from build123d import *

# Parameters (mm, degrees)
SKETCH2_R           = 35
SKETCH2_R_2         = 25.5
BOSS_EXTRUDE1_DEPTH = 3
SKETCH3_R           = 4
CUT_EXTRUDE1_DEPTH  = 5
SKETCH8_W           = 8
SKETCH8_H           = 8.160533217
CUT_EXTRUDE3_DEPTH  = 50.588305073
SKETCH9_R           = 1.65
CUT_EXTRUDE4_DEPTH  = 50.588305073


with BuildPart() as part:
    # Sketch2 → Boss-Extrude1 (new body)
    with BuildSketch(Plane.XY):
        Circle(SKETCH2_R)
        Circle(SKETCH2_R_2, mode=Mode.SUBTRACT)
    extrude(amount=BOSS_EXTRUDE1_DEPTH)

    # Sketch3 → Cut-Extrude1 (cut)
    with BuildSketch(Plane(origin=(0, 0, 0), x_dir=(-1, 0, 0), z_dir=(0, 0, -1))):
        with Locations((0, -33)):
            Circle(SKETCH3_R)
    extrude(amount=-CUT_EXTRUDE1_DEPTH, mode=Mode.SUBTRACT)

    # Sketch8 → Cut-Extrude3 (cut, through all)
    with BuildSketch(Plane.XY.offset(3)):
        with Locations((0, -37.080266608)):
            Rectangle(SKETCH8_W, SKETCH8_H)
    extrude(amount=-CUT_EXTRUDE3_DEPTH, mode=Mode.SUBTRACT)

    # Sketch9 → Cut-Extrude4 (cut, through all)
    with BuildSketch(Plane.XY.offset(3)):
        with Locations((30, 0)):
            Circle(SKETCH9_R)
        with Locations(Location((-30, 0, 0), (0, 0, 180))):
            Circle(SKETCH9_R)
    extrude(amount=-CUT_EXTRUDE4_DEPTH, mode=Mode.SUBTRACT)


solid = part.part
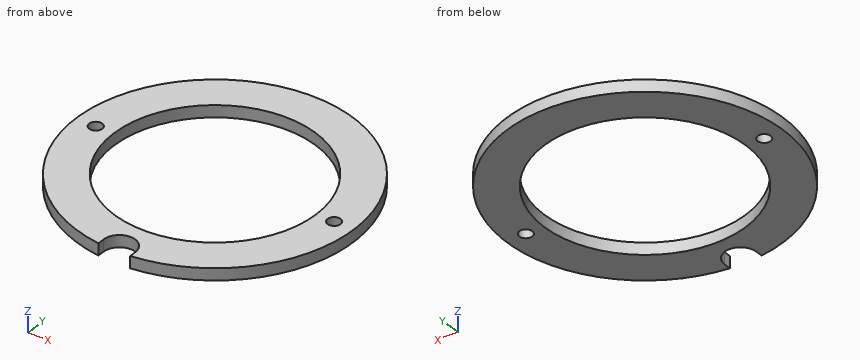
Design review of the part built by this model. Coordinates are the model's own, in mm. Round coordinates to 2 decimals unless told otherwise and drop trailing zeros. Write each loop counter-clockwise with the first axis right and the second up, starting at its lowest first coordinate (ties: lowest second). Pieces come first, ordered by that corner, then holes. Notation, with made-up numbers: (44.5, 84.25) - (94.5, 84.25) arc R23 cw to (94.5, 97.25) - close; hole circle Ø10 at (58, 86.5). An arc over 180 degrees is marked (long way). Use a Markdown table: item, result. Add a question column.
1. We need section B-B (x = 30). State the section outline as (y, z) points.
2. We need section A-A (z = 2.15). State the section outline as (x, y) points.
3. Clearance check with flat-ended pins moving along their axes: pin 1 (1 mm diameter, centred on y = -1, z = 2, fed in from -X); pin 2 (3 mm diameter, centred on x = -30, y = 0, fed in from -Z); pin 3 (1.5 mm diameter, centred on y = -20, z = 1, fed in from -X); pin 4 (1 mm diameter, centred on x = 10, z = 1, fed in from +Y). State where each tip first meets the part, or that it passes through.
4. We need section C-C (y = 0). State the section outline as (x, z) points.
5. We need section D-D (y = -15.5). State the section outline as (x, z) points.
6. Wall thickness on probe 1 along Y at (x, z) = (0, 1.8); probe 2 along Y at (x, z) = (13.5, 0.9); probe 3 along X at (y, z) = (-32, 2.65): over which ranges is each line inside the solid? List them lowest first.
Output:
| question | item | result |
|---|---|---|
| 1 | outline | (-18.03, 0) - (-1.65, 0) - (-1.65, 3) - (-18.03, 3) - close; (1.65, 0) - (18.03, 0) - (18.03, 3) - (1.65, 3) - close |
| 2 | outline | (-4, -34.77) - (-4, -33) arc R4 cw to (4, -33) - (4, -34.77) arc R35 ccw (long way) to start; hole circle Ø3.3 at (-30, 0); hole circle Ø51 at (0, 0); hole circle Ø3.3 at (30, 0) |
| 3 | pin 1 | stops at x = -35 |
| 3 | pin 2 | passes through |
| 3 | pin 3 | stops at x = -29.23 |
| 3 | pin 4 | stops at y = 33.69 |
| 4 | outline | (-35, 0) - (-31.65, 0) - (-31.65, 3) - (-35, 3) - close; (-28.35, 0) - (-25.5, 0) - (-25.5, 3) - (-28.35, 3) - close; (25.5, 0) - (28.35, 0) - (28.35, 3) - (25.5, 3) - close; (31.65, 0) - (35, 0) - (35, 3) - (31.65, 3) - close |
| 5 | outline | (-31.38, 0) - (-20.25, 0) - (-20.25, 3) - (-31.38, 3) - close; (20.25, 0) - (31.38, 0) - (31.38, 3) - (20.25, 3) - close |
| 6 | probe 1 | y = -29 to -25.5, 25.5 to 35 |
| 6 | probe 2 | y = -32.29 to -21.63, 21.63 to 32.29 |
| 6 | probe 3 | x = -14.18 to -3.87, 3.87 to 14.18 |
